```python
from build123d import *

# Parameters (mm, degrees)
BASE_PLATE_DEPTH         = 10
MOUNTING_FLANGE_SKETCH_W = 32.5
MOUNTING_FLANGE_SKETCH_H = 70
MOUNTING_FLANGE_DEPTH    = 10
FLANGE_LUGS_DEPTH        = 10
MOUNTING_HOLE_SKETCH_R   = 5
MOUNTING_HOLES_DEPTH     = 10
UPRIGHT_WEB_SKETCH_W     = 30
UPRIGHT_WEB_SKETCH_H     = 70
UPRIGHT_WEB_DEPTH        = 25
WEB_RELIEF_CUT_SKETCH_W  = 5
WEB_RELIEF_CUT_SKETCH_H  = 30
WEB_RELIEF_CUT_DEPTH     = 70
ROUNDED_ARM_DEPTH        = 70
BORE_BOSS_DEPTH          = 70
BORE_SKETCH_R            = 7.5
THROUGH_BORE_DEPTH       = 70


with BuildPart() as part:
    # Base Plate Sketch → Base Plate (new body)
    with BuildSketch(Plane.XY):
        with BuildLine():
            Line((0, 0), (47, 0))
            ThreePointArc((47, 0), (57.606601718, 4.393398282), (62, 15))
            Line((62, 15), (62, 25))
            Line((62, 25), (47, 25))
            ThreePointArc((47, 25), (37, 35), (47, 45))
            Line((47, 45), (62, 45))
            Line((62, 45), (62, 55))
            ThreePointArc((62, 55), (57.606601718, 65.606601718), (47, 70))
            Line((47, 70), (0, 70))
            Line((0, 70), (0, 0))
        make_face()
    extrude(amount=BASE_PLATE_DEPTH)

    # Mounting Flange Sketch → Mounting Flange (add)
    with BuildSketch(Plane.ZY):
        with Locations((26.25, 35)):
            Rectangle(MOUNTING_FLANGE_SKETCH_W, MOUNTING_FLANGE_SKETCH_H)
    extrude(amount=-MOUNTING_FLANGE_DEPTH)

    # Flange Lug Sketch → Flange Lugs (add)
    with BuildSketch(Plane(origin=(10, 0, 0), x_dir=(0, 0, -1), z_dir=(1, 0, 0))):
        with BuildLine():
            ThreePointArc((-45.5, 55.626136458), (-43.316699867, 53.78217355), (-42.5, 51.043560763))
            Line((-42.5, 51.043560763), (-42.5, 70))
            ThreePointArc((-42.5, 70), (-49.841797347, 64.032322328), (-45.5, 55.626136458))
        make_face()
        with BuildLine():
            Line((-42.5, 0), (-42.5, 18.956439237))
            ThreePointArc((-42.5, 18.956439237), (-43.316699867, 16.21782645), (-45.5, 14.373863542))
            ThreePointArc((-45.5, 14.373863542), (-49.841797347, 5.967677672), (-42.5, 0))
        make_face()
    extrude(amount=-FLANGE_LUGS_DEPTH)

    # Mounting Hole Sketch → Mounting Holes (cut)
    with BuildSketch(Plane(origin=(10, 0, 0), x_dir=(0, 0, -1), z_dir=(1, 0, 0))):
        with Locations((-42.5, 62.5)):
            Circle(MOUNTING_HOLE_SKETCH_R)
        with Locations((-42.5, 7.5)):
            Circle(MOUNTING_HOLE_SKETCH_R)
    extrude(amount=-MOUNTING_HOLES_DEPTH, mode=Mode.SUBTRACT)

    # Upright Web Sketch → Upright Web (add)
    with BuildSketch(Plane.ZY):
        with Locations((-15, 35)):
            Rectangle(UPRIGHT_WEB_SKETCH_W, UPRIGHT_WEB_SKETCH_H)
    extrude(amount=-UPRIGHT_WEB_DEPTH)

    # Web Relief Cut Sketch → Web Relief Cut (cut)
    with BuildSketch(Plane(origin=(0, 70, 0), x_dir=(1, 0, 0), z_dir=(0, 1, 0))):
        with Locations((22.5, 15)):
            Rectangle(WEB_RELIEF_CUT_SKETCH_W, WEB_RELIEF_CUT_SKETCH_H)
    extrude(amount=-WEB_RELIEF_CUT_DEPTH, mode=Mode.SUBTRACT)

    # Rounded Arm Sketch → Rounded Arm (add)
    with BuildSketch(Plane(origin=(0, 70, 0), x_dir=(1, 0, 0), z_dir=(0, 1, 0))):
        with BuildLine():
            Line((20, 0), (25, 0))
            ThreePointArc((25, 0), (21.464466094, 1.464466094), (20, 5))
            Line((20, 5), (20, 0))
        make_face()
    extrude(amount=-ROUNDED_ARM_DEPTH)

    # Bore Boss Sketch → Bore Boss (add)
    with BuildSketch(Plane(origin=(0, 70, 0), x_dir=(1, 0, 0), z_dir=(0, 1, 0))):
        with BuildLine():
            Line((0, 30), (20, 30))
            ThreePointArc((20, 30), (10, 40), (0, 30))
        make_face()
    extrude(amount=-BORE_BOSS_DEPTH)

    # Bore Sketch → Through Bore (cut)
    with BuildSketch(Plane(origin=(0, 70, 0), x_dir=(1, 0, 0), z_dir=(0, 1, 0))):
        with Locations(Location((10, 30, 0), (0, 0, 270))):
            Circle(BORE_SKETCH_R)
    extrude(amount=-THROUGH_BORE_DEPTH, mode=Mode.SUBTRACT)


solid = part.part
```
Verification items for the finished model (mm, model axes). A direction names the side the tool comes from. Coordinates: 2 decimals unless noted, no trailing zeros. Loops run counter-clockwise (first coordinate to the right, second up) from the corner with the lowest first, then second, coordinate; pieces in that order, holes last. Notation, with made-up numbers: (36, 72.25) -> (41, 72.25) arc R19 cw to (41, 80.25) -> close; hole circle Ø6 at (77, 77.5). An arc over 180 degrees is marked (long way). Answer in a Markdown table with one row per item. Add a question column.
1. Access from +Z, -Z, +X, -X, +Y, -Y to the whole of each face (thin tool, end or side, straight path). Record for faces 5 (the face through (20, 35, -17)), 6 (the face through (57.49, 4.28, 4.93)), 7 (the face through (30, 35, 10)), 8 (the face through (54, 45, 5)), 9 (the face through (5.07, 53.82, 43.34)).
2. Depth check by flat-ended pin: P1, Ø11, axis at x = 51, z = 4.5, coming from the -Y side; P2, Ø6, axis at y = 62.5, z = 42.5, coming from the +X side; P3, Ø4, axis at y = 17, z = -3.5, coming from the +X side; P4, Ø10, axis at x = 16, y = 55, coming from the -Z side. Enter the tip coordinate at first touch or a pass-through.
3. Section check D-D, the plane y = 47.5. Enter the section's corners in (x, z).
4. Draft check along Z on faces 1 (the face through (57.72, 65.49, 4.93)), 2 (the face through (10, 35, -40)), 3 (the face through (2.68, 35.49, -31.63)), 4 (the face through (5.07, 6.11, 49.87)). Enter one of: +Z half, -Z half, draft (parallel to the pull), parting line (faces both ways), or undercut.
5. Section check A-A, the plane y = 35. Enter the section's corners in (x, z), then the cut area to 3 significant figures.
6. Section check B-B, the plane x = 52. Enter the section's corners in (y, z).
7. Material ranges on probe 1 along Y at (x, z) = (5, 42); probe 2 along Z at (x, y) = (5, 62); probe 3 along Z at (x, y) = (4, 62), recorded low to high. Write a range as [from, to].
8. Section check C-C, the plane y = 62.5. Enter the section's corners in (x, z).
Derived:
| question | item | result |
|---|---|---|
| 1 | face 5 | -Z, +X, +Y, -Y |
| 1 | face 6 | +Z, -Z, +X, -Y |
| 1 | face 7 | +Z, +X, +Y, -Y |
| 1 | face 8 | +Z, -Z, +X |
| 1 | face 9 | +Z, +X, -X |
| 2 | P1 | stops at y = 0 |
| 2 | P2 | passes through |
| 2 | P3 | stops at x = 21.43 |
| 2 | P4 | stops at z = -39.95 |
| 3 | outline | (0, -30) arc R10 ccw to (20, -30) -> (20, -5) arc R5 cw to (25, 0) -> (62, 0) -> (62, 10) -> (10, 10) -> (10, 42.5) -> (0, 42.5) -> close; hole circle Ø15 at (10, -30) |
| 4 | face 1 | draft |
| 4 | face 2 | -Z half |
| 4 | face 3 | undercut |
| 4 | face 4 | +Z half |
| 5 | outline | (0, -30) arc R10 ccw to (20, -30) -> (20, -5) arc R5 cw to (25, 0) -> (37, 0) -> (37, 10) -> (10, 10) -> (10, 42.5) -> (0, 42.5) -> close; hole circle Ø15 at (10, -30) |
| 5 | area | 1,280 mm² |
| 6 | outline | (0.86, 0) -> (25, 0) -> (25, 10) -> (0.86, 10) -> close; (45, 0) -> (69.14, 0) -> (69.14, 10) -> (45, 10) -> close |
| 7 | probe 1 | y = [0, 2.53], [12.47, 57.53], [67.47, 70] |
| 7 | probe 2 | z = [-38.66, -35.59], [-24.41, 37.53], [47.47, 49.98] |
| 7 | probe 3 | z = [-38, -34.5], [-25.5, 37.53], [47.47, 49.98] |
| 8 | outline | (0, -30) arc R10 ccw to (20, -30) -> (20, -5) arc R5 cw to (25, 0) -> (59.99, 0) -> (59.99, 10) -> (10, 10) -> (10, 37.5) -> (0, 37.5) -> close; (0, 47.5) -> (10, 47.5) -> (10, 50) -> (0, 50) -> close; hole circle Ø15 at (10, -30) |
